```python
from build123d import *

# Parameters (mm, degrees)
SKETCH1_R           = 35
SKETCH1_R_2         = 30
BOSS_EXTRUDE1_DEPTH = 30
SKETCH2_R           = 45
SKETCH2_R_2         = 30
BOSS_EXTRUDE2_DEPTH = 5
SKETCH3_R           = 2.5
CUT_EXTRUDE1_DEPTH  = 50
CHAMFER1_SIZE       = 1


with BuildPart() as part:
    # Sketch1 → Boss-Extrude1 (new body)
    with BuildSketch(Plane.XY):
        Circle(SKETCH1_R)
        Circle(SKETCH1_R_2, mode=Mode.SUBTRACT)
    extrude(amount=BOSS_EXTRUDE1_DEPTH)

    # Sketch2 → Boss-Extrude2 (add)
    with BuildSketch(Plane.XY.offset(30)):
        Circle(SKETCH2_R)
        Circle(SKETCH2_R_2, mode=Mode.SUBTRACT)
    extrude(amount=BOSS_EXTRUDE2_DEPTH)

    # Sketch3 → Cut-Extrude1 (cut)
    with BuildSketch(Plane(origin=(0, 0, 30), x_dir=(-1, 0, 0), z_dir=(0, 0, -1))):
        with Locations((41, 0)):
            Circle(SKETCH3_R)
        with Locations((-20.5, -35.507041555)):
            Circle(SKETCH3_R)
        with Locations((-20.5, 35.507041555)):
            Circle(SKETCH3_R)
    extrude(amount=-CUT_EXTRUDE1_DEPTH, mode=Mode.SUBTRACT)

    # Chamfer1
    chamfer1_edges = [part.edges().sort_by_distance(p)[0] for p in [
        (-30, 0, 35),
        (-35, 0, 0),
        (-30, 0, 0),
    ]]
    chamfer(chamfer1_edges, length=CHAMFER1_SIZE)


solid = part.part
```
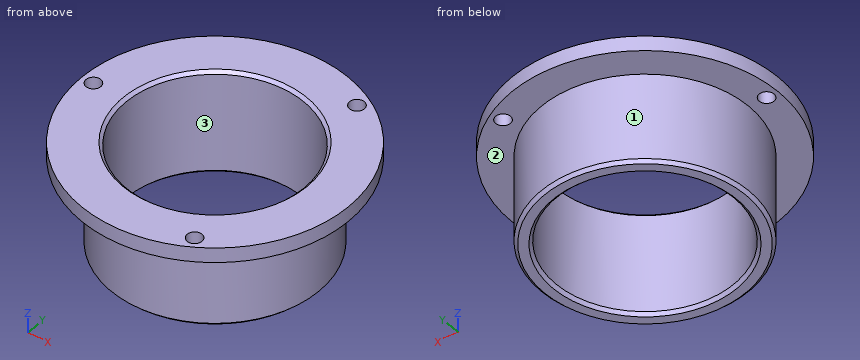
Geometry: final body of the model. Coordinates: model frame, mm. Face numbers are marked on the shaded views. Round coordinates to 2 decimals unless told otherwise and drop trailing zeros. Order: outer loops, then holes, each group sorted by start corner. A loop starts at its lowest first (then second) coordinate and runs counter-clockwise, first axis right, second up. Notation, with made-up numbers: (23.25, 18.5) - (47.25, 18.5) arc R34 cw to (47.25, 55.5) - close; hole circle Ø7 at (26.25, 5.25). An arc over 180 degrees is marked (long way). Use CSV: the item, a comma, the result in double quotes. Start each with the question number.
Q1. Section query C-C (z = 16). Return loops of the section in (x, y).
Q2. Material intervals for line 1 along Y through (x, z) = (-1, 33); line 2 along Y through (x, z) = (20.5, 32.6); line 3 along Y through (x, z) = (0, 4), sorted ascending. Write a range as from..to.
Q3. First-contact query: pin 1 (6 mm diameter, centred on y = -26, z = 6.5, fed in from -X); pin 2 (8 mm diameter, centred on x = -18, z = 17, fed in from -Y); pin 3 (8 mm diameter, centred on x = 20.5, y = 35.51, fed in from -Z). Flat tips, straight axial feed; report the tip coordinate or a pass-through.
Q4. Section query A-A (y = 0). Return loops of the section in (x, z).
Q5. Section query B-B (x = 0). Return loops of the section in (y, z).
Q6. Mould query, pull axis Y, two halves, no side actions, for the marked faces 1, 2 and 3. Classes: +Y half, -Y half, draft (parallel to the pull), parting line (faces both ways), or undercut.
Q7. Section query D-D (x = -41). Return loops of the section in (y, z), and give its area (3 significant figures).
Result set:
1,outline,"circle Ø70 at (0, 0); hole circle Ø60 at (0, 0)"
2,line 1,"y = -44.99..-29.98, 29.98..44.99"
2,line 2,"y = -40.06..-38.01, -33.01..-21.9, 21.9..33.01, 38.01..40.06"
2,line 3,"y = -35..-30, 30..35"
3,pin 1,"stops at x = -26.38"
3,pin 2,"stops at y = -32.08"
3,pin 3,"stops at z = 30"
4,outline,"(-45, 30) - (-43.5, 30) - (-43.5, 35) - (-45, 35) - close; (-38.5, 30) - (-35, 30) - (-35, 1) - (-34, 0) - (-31, 0) - (-30, 1) - (-30, 34) - (-31, 35) - (-38.5, 35) - close; (30, 1) - (31, 0) - (34, 0) - (35, 1) - (35, 30) - (45, 30) - (45, 35) - (31, 35) - (30, 34) - close"
5,outline,"(-45, 30) - (-35, 30) - (-35, 1) - (-34, 0) - (-31, 0) - (-30, 1) - (-30, 34) - (-31, 35) - (-45, 35) - close; (30, 1) - (31, 0) - (34, 0) - (35, 1) - (35, 30) - (45, 30) - (45, 35) - (31, 35) - (30, 34) - close"
6,face 1,"parting line"
6,face 2,"draft"
6,face 3,"undercut"
7,outline,"(-18.55, 30) - (-2.5, 30) - (-2.5, 35) - (-18.55, 35) - close; (2.5, 30) - (18.55, 30) - (18.55, 35) - (2.5, 35) - close"
7,area,"160 mm2"
